```python
from build123d import *

# Parameters (mm, degrees)
SKETCH1_R           = 159.746139417
SKETCH1_R_2         = 1.5
SKETCH1_R_3         = 137.746139417
BOSS_EXTRUDE1_DEPTH = 6


with BuildPart() as part:
    # Sketch1 → Boss-Extrude1 (new body)
    with BuildSketch(Plane.XY):
        Circle(SKETCH1_R)
        with BuildLine():
            ThreePointArc((-91.383895087, -127.663556737), (-111.015764646, -111.015764646), (-127.663556737, -91.383895087))
            ThreePointArc((-127.663556737, -91.383895087), (-127.684062187, -86.718774861), (-123.01894196, -86.698269411))
            ThreePointArc((-123.01894196, -86.698269411), (-106.419570569, -106.419570569), (-86.698269411, -123.01894196))
            ThreePointArc((-86.698269411, -123.01894196), (-86.718774861, -127.684062187), (-91.383895087, -127.663556737))
        make_face(mode=Mode.SUBTRACT)
        with Locations((-8.7, -157.446139417)):
            Circle(SKETCH1_R_2, mode=Mode.SUBTRACT)
        with Locations((-8.7, -140.046139417)):
            Circle(SKETCH1_R_2, mode=Mode.SUBTRACT)
        with Locations((-157.446139417, -8.7)):
            Circle(SKETCH1_R_2, mode=Mode.SUBTRACT)
        with Locations((-140.046139417, -8.7)):
            Circle(SKETCH1_R_2, mode=Mode.SUBTRACT)
        with Locations((8.7, -157.446139417)):
            Circle(SKETCH1_R_2, mode=Mode.SUBTRACT)
        with Locations((8.7, -140.046139417)):
            Circle(SKETCH1_R_2, mode=Mode.SUBTRACT)
        with BuildLine():
            ThreePointArc((127.663556737, -91.383895087), (111.015764646, -111.015764646), (91.383895087, -127.663556737))
            ThreePointArc((91.383895087, -127.663556737), (86.718774861, -127.684062187), (86.698269411, -123.01894196))
            ThreePointArc((86.698269411, -123.01894196), (106.419570569, -106.419570569), (123.01894196, -86.698269411))
            ThreePointArc((123.01894196, -86.698269411), (127.684062187, -86.718774861), (127.663556737, -91.383895087))
        make_face(mode=Mode.SUBTRACT)
        with Locations((140.046139417, -8.7)):
            Circle(SKETCH1_R_2, mode=Mode.SUBTRACT)
        with Locations((157.446139417, -8.7)):
            Circle(SKETCH1_R_2, mode=Mode.SUBTRACT)
        with Locations((-157.446139417, 8.7)):
            Circle(SKETCH1_R_2, mode=Mode.SUBTRACT)
        with Locations((-140.046139417, 8.7)):
            Circle(SKETCH1_R_2, mode=Mode.SUBTRACT)
        with BuildLine():
            ThreePointArc((-127.663556737, 91.383895087), (-111.015764646, 111.015764646), (-91.383895087, 127.663556737))
            ThreePointArc((-91.383895087, 127.663556737), (-86.718774861, 127.684062187), (-86.698269411, 123.01894196))
            ThreePointArc((-86.698269411, 123.01894196), (-106.419570569, 106.419570569), (-123.01894196, 86.698269411))
            ThreePointArc((-123.01894196, 86.698269411), (-127.684062187, 86.718774861), (-127.663556737, 91.383895087))
        make_face(mode=Mode.SUBTRACT)
        with Locations((-8.7, 140.046139417)):
            Circle(SKETCH1_R_2, mode=Mode.SUBTRACT)
        with Locations((-8.7, 157.446139417)):
            Circle(SKETCH1_R_2, mode=Mode.SUBTRACT)
        Circle(SKETCH1_R_3, mode=Mode.SUBTRACT)
        with Locations((140.046139417, 8.7)):
            Circle(SKETCH1_R_2, mode=Mode.SUBTRACT)
        with Locations((157.446139417, 8.7)):
            Circle(SKETCH1_R_2, mode=Mode.SUBTRACT)
        with Locations((8.7, 140.046139417)):
            Circle(SKETCH1_R_2, mode=Mode.SUBTRACT)
        with Locations((8.7, 157.446139417)):
            Circle(SKETCH1_R_2, mode=Mode.SUBTRACT)
        with BuildLine():
            ThreePointArc((91.383895087, 127.663556737), (111.015764646, 111.015764646), (127.663556737, 91.383895087))
            ThreePointArc((127.663556737, 91.383895087), (127.684062187, 86.718774861), (123.01894196, 86.698269411))
            ThreePointArc((123.01894196, 86.698269411), (106.419570569, 106.419570569), (86.698269411, 123.01894196))
            ThreePointArc((86.698269411, 123.01894196), (86.718774861, 127.684062187), (91.383895087, 127.663556737))
        make_face(mode=Mode.SUBTRACT)
    extrude(amount=BOSS_EXTRUDE1_DEPTH)


solid = part.part
```
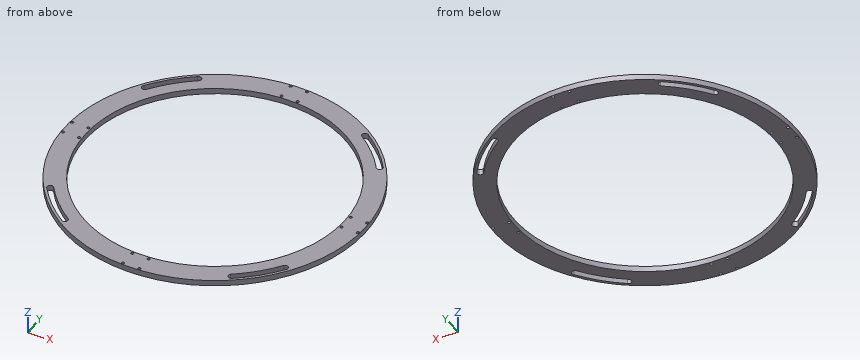
Source: CAD feature listing. Evaluate the final solid. Frame: model axes, mm. Round coordinates to 2 decimals unless told otherwise and drop trailing zeros. Order: outer loops, then holes, each group sorted by start corner. A loop starts at its lowest first (then second) coordinate and runs counter-clockwise, first axis right, second up. Notation, with made-up numbers: (11.25, 45) -> (24.25, 45) arc R38 cw to (24.25, 83) -> close; hole circle Ø6 at (-9, 41). An arc over 180 degrees is marked (long way). One line per item, written item: value. Start each with the question number.
Q1. Section query C-C (z = 1.55). Give the number of separate pieces and of enclosed holes in the cut face, plus the area to 3 significant figures.
Q2. Pin query (flat end, axial travel): pin 1 (2.5 mm diameter, centred on x = 157.45, y = -8.7, fed in from +Z); pin 2 (1.5 mm diameter, centred on y = 102, z = 5, fed in from +X); pin 3 (3 mm diameter, centred on y = -52.5, z = 5, fed in from -X); pin 4 (2 mm diameter, centred on y = -51.5, z = 2, fed in from +X). Return the tip coordinate at first contact, or that it passes through.
Q3. Material intervals for probe 1 along Y at (x, z) = (0, 4.1); probe 2 along Y at (x, z) = (100.5, 1.6); probe 3 along Y at (x, z) = (-8.7, 2.85), sorted ascending.
Q4. Section query A-A (x = 0). Return the cut outline in (y, z), plus the area to 3 significant figures.
Findings below:
1. separate pieces: 1
1. enclosed holes: 21
1. area: 19,000 mm²
2. pin 1: through
2. pin 2: x = 123.56
2. pin 3: x = -151.39
2. pin 4: x = 151.55
3. probe 1: -159.75 to -137.75, 137.75 to 159.75
3. probe 2: -124.17 to -120.62, -112.03 to -94.2, 94.2 to 112.03, 120.62 to 124.17
3. probe 3: -159.51 to -158.95, -155.95 to -141.55, -138.55 to -137.47, 137.47 to 138.55, 141.55 to 155.95, 158.95 to 159.51
4. outline: (-159.75, 0) -> (-137.75, 0) -> (-137.75, 6) -> (-159.75, 6) -> close; (137.75, 0) -> (159.75, 0) -> (159.75, 6) -> (137.75, 6) -> close
4. area: 264 mm²
